Check sheet for the drawn part. Datum: minimum x, y, z corner. Units: mm. A direction names the side the tool comes from. Give positions to 0.01 mm unless a question says otherwise; leave off trailing zeros. Order: outer loops, then holes, each group sorted by start corner. A loop starts at its lowest first (then second) coordinate and runs counter-clockwise, first axis right, second up.
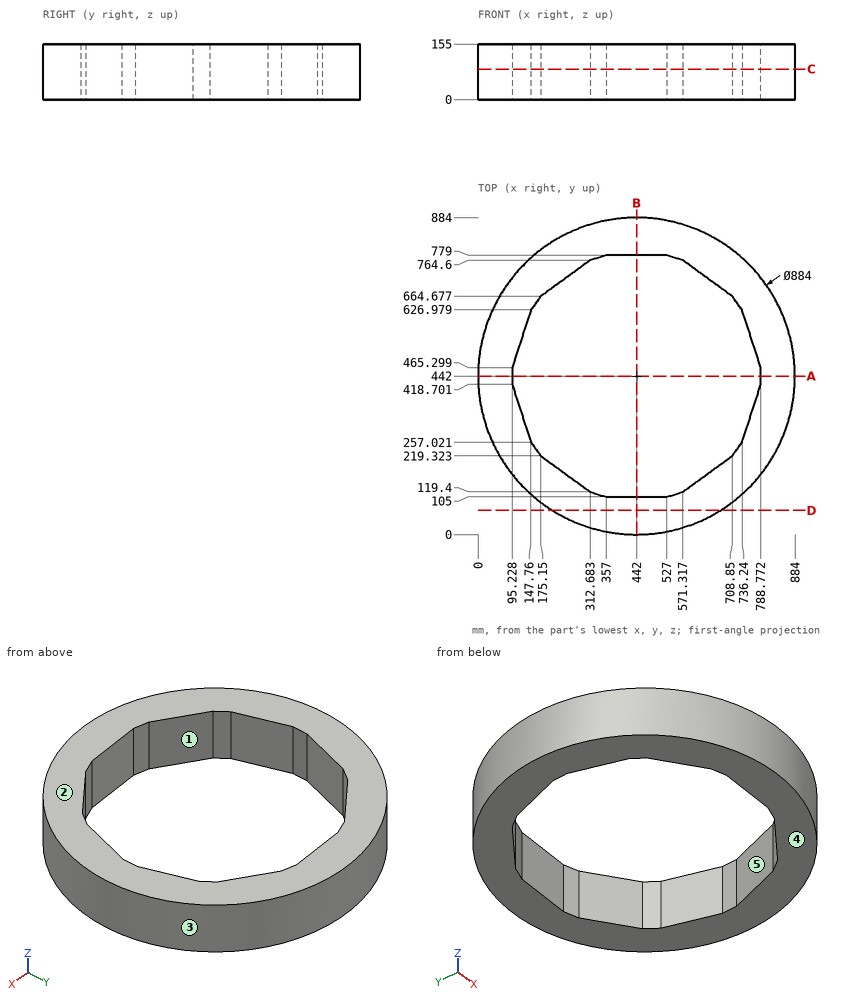
Q1. Sectioned sample at A-A, the plane y = 442. Record the cut outline in (x, z), plus the area to 3 significant figures.
Q2. Sectioned sample at D-D, the plane y = 67.5. Record the cut outline in (x, z), plus the area to 3 significant figures.
Q3. Tool access check on the marked faces 4 and 5. Record the directions out of +Z, -Z, +X, -X, +Y, -Y that give a thin tool (end or side, any length) a straight path to the whole face; none if there is none.
Q4. Sectioned sample at C-C, the plane z = 85. Record the cut outline in (x, y).
Q5. Sectioned sample at B-B, the plane x = 442. Record the cut outline in (y, z).
Q6. Draft check along X on the marked faces 1, 2 and 3. Enter one of: pulls with the +X half, pulls with the -X half, needs draft (parallel to the pull), parting line crosses it, or undercut.
Q7. Go/stop test with flat-tipped pins: P1, Ø10, axis at y = 557, z = 32.5, coming from the +X side; P2, Ø23.5, axis at y = 448.5, z = 59, coming from the +X side; P3, Ø1.5, axis at x = 212.5, z = 102.5, coming from the +Y side; P4, Ø1.5, axis at y = 417, z = 22, coming from the -X side. Record where each tip stops, or that it passes through.
Q8. Material ranges on line 1 (Y direction, x = 432, z = 147); line 2 (Y direction, x = 439.5, z = 40.5); line 3 (X direction, y = 628, z = 73.5), recorded low to high.
Filled in:
1. outline: (0, 0) - (95.23, 0) - (95.23, 155) - (0, 155) - close; (788.77, 0) - (884, 0) - (884, 155) - (788.77, 155) - close
1. area: 29,500 mm2
2. outline: (207.24, 0) - (676.76, 0) - (676.76, 155) - (207.24, 155) - close
2. area: 72,800 mm2
3. face 4: -Z, +X, -X, +Y, -Y
3. face 5: +Z, -Z
4. outline: circle Ø884 at (442, 442); hole (95.23, 418.7) - (147.76, 257.02) - (175.15, 219.32) - (312.68, 119.4) - (357, 105) - (527, 105) - (571.32, 119.4) - (708.85, 219.32) - (736.24, 257.02) - (788.77, 418.7) - (788.77, 465.3) - (736.24, 626.98) - (708.85, 664.68) - (571.32, 764.6) - (527, 779) - (357, 779) - (312.68, 764.6) - (175.15, 664.68) - (147.76, 626.98) - (95.23, 465.3) - close
5. outline: (0, 0) - (105, 0) - (105, 155) - (0, 155) - close; (779, 0) - (884, 0) - (884, 155) - (779, 155) - close
6. face 1: undercut
6. face 2: needs draft
6. face 3: parting line crosses it
7. P1: stops at x = 870.09
7. P2: stops at x = 884
7. P3: stops at y = 820.2
7. P4: stops at x = 0.67
8. line 1: y = 0.11 to 105, 779 to 883.89
8. line 2: y = 0.01 to 105, 779 to 883.99
8. line 3: x = 41.04 to 148.5, 735.5 to 842.96
